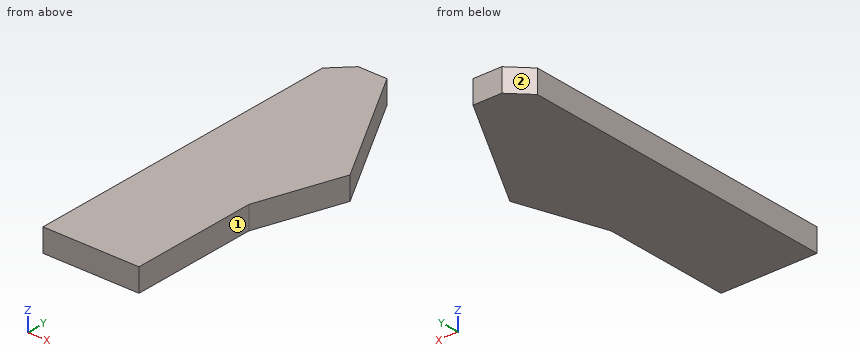
from build123d import *

# Parameters (mm, degrees)
BOSS_EXTRUDE1_DEPTH = 6
CHAMFER1_SIZE       = 10


with BuildPart() as part:
    # Sketch1 → Boss-Extrude1 (new, symmetric)
    with BuildSketch(Plane.XY):
        Polygon((0, 0), (0, 180), (25, 180), (64.770332896, 111.11576279), (50, 66.792003178), (50, 0), align=None)
    extrude(amount=BOSS_EXTRUDE1_DEPTH, both=True)

    # Chamfer1
    chamfer1_edges = [part.edges().sort_by_distance(p)[0] for p in [
        (0, 180, 0),
    ]]
    chamfer(chamfer1_edges, length=CHAMFER1_SIZE)


solid = part.part
The model under review builds one solid part; all positions refer to its coordinate system, in mm. Face numbers are marked on the shaded views. A direction names the side the tool comes from. Round coordinates to 2 decimals unless told otherwise and drop trailing zeros. Loops run counter-clockwise (first coordinate to the right, second up) from the corner with the lowest first, then second, coordinate; pieces in that order, holes last. Notation, with made-up numbers: M 15,-17 L 55,-17 A25 ccw 55,18 Z; hole C -25,71 d1. An arc over 180 degrees is marked long. Answer as CSV lines item,"result". Start each with the question number.
Item 1: Consider section B-B (x = 40). Write out the cut boundary in (y, z).
Item 2: Consider section A-A (z = -1). Write out the cut boundary in (x, y).
Item 3: Consider section C-C (y = 168). Write out the cut boundary in (x, z), then the cut area to 3 significant figures.
Item 4: Insertion check: P1, Ø5, axis at x = 7, z = -3, coming from the +Y side; P2, Ø1.5, axis at y = 117, z = 0, coming from the +X side; P3, Ø1, axis at x = 53.5, z = 0, coming from the +Y side. Each pin has a flat end and moves straight along its axis. Give the tip position at first contact, or say it passes through.
Item 5: For the marked faces 1 and 2, list the 3-axis set-ups (+Z, -Z, +X, -X, +Y, -Y) from which the entire face can be reached by the end or side of a thin tool; tool diameter is ignored.
Item 6: Wall thickness on line 1 (X direction, y = 36, z = -4.75); line 2 (Y direction, x = 43.5, z = -2.75); line 3 (X direction, y = 110, z = 0.75): over which ranges is each line inside the solid? List them lowest first. Write a range as [from, to].
Answer:
1,outline,"M 0,-6 L 154.02,-6 L 154.02,6 L 0,6 Z"
2,outline,"M 0,0 L 50,0 L 50,66.79 L 64.77,111.12 L 25,180 L 10,180 L 0,170 Z"
3,outline,"M 0,-6 L 31.93,-6 L 31.93,6 L 0,6 Z"
3,area,"383 mm^2"
4,P1,"stops at y = 179.5"
4,P2,"stops at x = 61.81"
4,P3,"stops at y = 131.5"
5,face 1,"+Z, -Z, +X, -Y"
5,face 2,"+Z, -Z, -X, +Y"
6,line 1,"x = [0, 50]"
6,line 2,"y = [0, 147.96]"
6,line 3,"x = [0, 64.4]"
